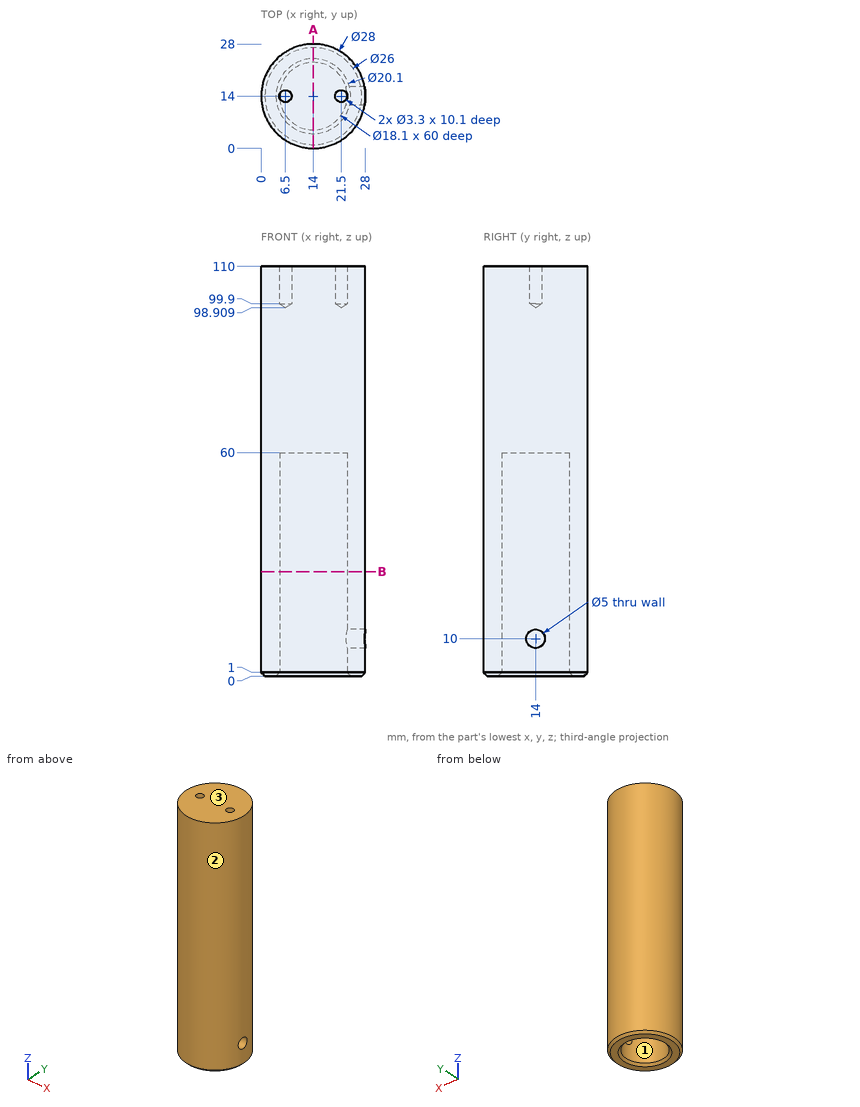
Check sheet for the drawn part. Datum: minimum x, y, z corner. Units: mm. Give positions to 0.01 mm unless a question says otherwise; leave off trailing zeros. Write each loop counter-clockwise with the first axis right and the second up, starting at its lowest first coordinate (ties: lowest second). Pieces come first, ordered by that corner, then holes. Notation, with made-up numbers: (-11, 71.25) - (41, 71.25) arc R25 ccw to (41, 106.25) - close; hole circle Ø4 at (-25, 53.25). An arc over 180 degrees is marked (long way). Put each result on its own line as item: value.
1. Sectioned sample at B-B, the plane z = 28. Enter the section's corners in (x, y).
Ans:
outline: circle Ø28 at (14, 14); hole circle Ø18.1 at (14, 14)
2. Draft check along X on the marked faces 1, 2 and 3. Enter one of: +X half, -X half, draft (parallel to the pull), parting line (faces both ways), or undercut.
Ans:
face 1: undercut
face 2: parting line
face 3: draft
3. Sectioned sample at A-A, the plane x = 14. Enter the section's corners in (y, z), plus the area to 3 significant figures.
Ans:
outline: (0, 1) - (1, 0) - (3.95, 0) - (4.95, 1) - (4.95, 60) - (23.05, 60) - (23.05, 1) - (24.05, 0) - (27, 0) - (28, 1) - (28, 110) - (0, 110) - close
area: 1,990 mm²
4. Go/stop test with flat-tipped pins: pin 1 (1.5 mm diameter, centred on y = 8.5, z = 35.5, fed in from +X); pin 2 (9 mm diameter, centred on x = 14, y = 17, fed in from -Z); pin 3 (2 mm diameter, centred on y = 5.5, z = 84.5, fed in from +X). Record where each tip stops, or that it passes through.
Ans:
pin 1: stops at x = 27.17
pin 2: stops at z = 60
pin 3: stops at x = 25.82
5. Thickness scan on line 1 (Y direction, x = 14, z = 15); line 2 (Y direction, x = 6.5, z = 105.25); line 3 (Z direction, x = 15.25, y = 18.75). Record the ranges inside material, lowest first.
Ans:
line 1: y = 0 to 4.95, 23.05 to 28
line 2: y = 2.18 to 12.35, 15.65 to 25.82
line 3: z = 60 to 110
